The model under review builds one solid part; all positions refer to its coordinate system, in mm. A direction names the side the tool comes from. Coordinates: 2 decimals unless noted, no trailing zeros. Order: outer loops, then holes, each group sorted by start corner. A loop starts at its lowest first (then second) coordinate and runs counter-clockwise, first axis right, second up. Notation, with made-up numbers: (77, -6.5) -> (105, -6.5) arc R24 ccw to (105, 12.5) -> close; hole circle Ø3 at (-5.75, -7.5). An arc over 180 degrees is marked (long way). Use one line per item in the form item = value. Start each with the question number.
(1) Take a section at C-C (y = -4). State the section outline as (x, z) points, then the cut area to 3 significant figures.
(2) Mouldability with a two-part tool opening along Y and no side actions: class faces 4 (the flat face through (3, 17, -10)), 5 (the flat face through (2, 25, 0)), 6 (the cylindrical face through (-178.97, 0.93, 7.54)), 7 (the cylindrical face through (-190.943, 1.728, 0.14)) as +Y half, -Y half, draft (parallel to the pull), parting line (faces both ways), or undercut.
(3) Wall thickness on line 1 along Y through (x, z) = (76, 1.5); line 2 along X through (y, z) = (-1.5, -1.25); line 3 along Y through (x, z) = (-9, -9): over which ranges is each line inside the solid? List them lowest first.
(4) For faces 1 (the flat face through (2, -31.598, 0)), 2 (the cylindrical face through (189.945, 1.661, 0.07)), 3 (the cylindrical face through (-178.97, 0.93, -7.46)), list the 3-axis set-ups (+Z, -Z, +X, -X, +Y, -Y) from which the entire face can be reached by the end or side of a thin tool; tool diameter is ignored.
(5) Take a section at D-D (y = 21.5). State the section outline as (x, z) points.
(6) Take a section at A-A (x = 40.5). State the section outline as (y, z) points, then the cut area to 3 significant figures.
(7) Take a section at B-B (z = -1.25). State the section outline as (x, y) points (3 decimals), then the cut area to 3 significant figures.
(8) Insertion check: pin 1 Ø12 at (y, z) = (10.5, -7) entering from -X; pin 2 Ø1.5 at (y, z) = (11.5, 3.5) entering from +X; pin 3 Ø1 at (y, z) = (-7, -5.5) entering from +X. Each pin has a flat end and moves straight along its axis. Give the tip position at first contact, or say it passes through.
```python
from build123d import *

# Parameters (mm, degrees)
BOSS_EXTRUDE1_DEPTH = 10
CUT_EXTRUDE1_DEPTH  = 5


with BuildPart() as part:
    # Sketch2 → Boss-Extrude1 (new, symmetric)
    with BuildSketch(Plane.XY):
        with BuildLine():
            Line((-165, 26), (165, 26))
            ThreePointArc((165, 26), (190.90106215, 2.266049311), (169.514852619, -25.605001578))
            Line((169.514852619, -25.605001578), (135.524931981, -31.598341659))
            Line((135.524931981, -31.598341659), (-135.524931981, -31.598341659))
            Line((-135.524931981, -31.598341659), (-169.514852619, -25.605001578))
            ThreePointArc((-169.514852619, -25.605001578), (-190.90106215, 2.266049311), (-165, 26))
        make_face()
        with BuildLine():
            Line((-165, 14), (165, 14))
            ThreePointArc((165, 14), (178.946725773, 1.220180398), (167.431074487, -13.787308542))
            Line((167.431074487, -13.787308542), (134.475068019, -19.598341659))
            Line((134.475068019, -19.598341659), (-134.475068019, -19.598341659))
            Line((-134.475068019, -19.598341659), (-167.431074487, -13.787308542))
            ThreePointArc((-167.431074487, -13.787308542), (-178.946725773, 1.220180398), (-165, 14))
        make_face(mode=Mode.SUBTRACT)
    extrude(amount=BOSS_EXTRUDE1_DEPTH, both=True)

    # Sketch8 → Cut-Extrude1 (cut, symmetric)
    with BuildSketch(Plane.XY):
        with BuildLine():
            Line((135.437443318, -30.598341659), (169.341204442, -24.620193825))
            ThreePointArc((169.341204442, -24.620193825), (189.904867452, 2.178893569), (165, 25))
            Line((165, 25), (-165, 25))
            ThreePointArc((-165, 25), (-189.904867452, 2.178893569), (-169.341204442, -24.620193825))
            Line((-169.341204442, -24.620193825), (-135.437443318, -30.598341659))
            Line((-135.437443318, -30.598341659), (135.437443318, -30.598341659))
        make_face()
    extrude(amount=CUT_EXTRUDE1_DEPTH, both=True, mode=Mode.SUBTRACT)


solid = part.part
```
Findings:
q1.outline = (-190.69, -10) -> (-178.42, -10) -> (-178.42, -5) -> (-189.68, -5) -> (-189.68, 5) -> (-178.42, 5) -> (-178.42, 10) -> (-190.69, 10) -> close; (178.42, -10) -> (190.69, -10) -> (190.69, 10) -> (178.42, 10) -> (178.42, 5) -> (189.68, 5) -> (189.68, -5) -> (178.42, -5) -> close
q1.area = 266 mm²
q2.face_4 = draft
q2.face_5 = undercut
q2.face_6 = undercut
q2.face_7 = parting line
q3.line_1 = -31.6 to -30.6, 25 to 26
q3.line_2 = -190.96 to -189.95, 189.95 to 190.96
q3.line_3 = -31.6 to -19.6, 14 to 26
q4.face_1 = +Z, -Z, +X, -X, -Y
q4.face_2 = none
q4.face_3 = +Z, -Z
q5.outline = (-179.62, -10) -> (179.62, -10) -> (179.62, 10) -> (-179.62, 10) -> close; hole (-177.76, -5) -> (177.76, -5) -> (177.76, 5) -> (-177.76, 5) -> close
q6.outline = (-31.6, -10) -> (-19.6, -10) -> (-19.6, -5) -> (-30.6, -5) -> (-30.6, 5) -> (-19.6, 5) -> (-19.6, 10) -> (-31.6, 10) -> close; (14, -10) -> (26, -10) -> (26, 10) -> (14, 10) -> (14, 5) -> (25, 5) -> (25, -5) -> (14, -5) -> close
q6.area = 260 mm²
q7.outline = (-169.515, -25.605) -> (-135.525, -31.598) -> (135.525, -31.598) -> (169.515, -25.605) arc R26 ccw to (165, 26) -> (-165, 26) arc R26 ccw to start; hole (-169.341, -24.62) -> (-135.437, -30.598) -> (135.437, -30.598) -> (169.341, -24.62) arc R25 ccw to (165, 25) -> (-165, 25) arc R25 ccw to start
q7.area = 821 mm²
q8.pin_1 = -190.61
q8.pin_2 = 188.67
q8.pin_3 = 190.17
